For this review, take the finished solid that the model builds, in its own axes (mm). Coordinates: 2 decimals unless noted, no trailing zeros. Loops run counter-clockwise (first coordinate to the right, second up) from the corner with the lowest first, then second, coordinate; pieces in that order, holes last. Notation, with made-up numbers: (55.5, -18.5) -> (70.5, -18.5) arc R17 ccw to (70.5, -11.5) -> close; hole circle Ø5 at (-28.75, -33.75). An arc over 180 degrees is marked (long way). Answer in a Markdown table with one row per item.
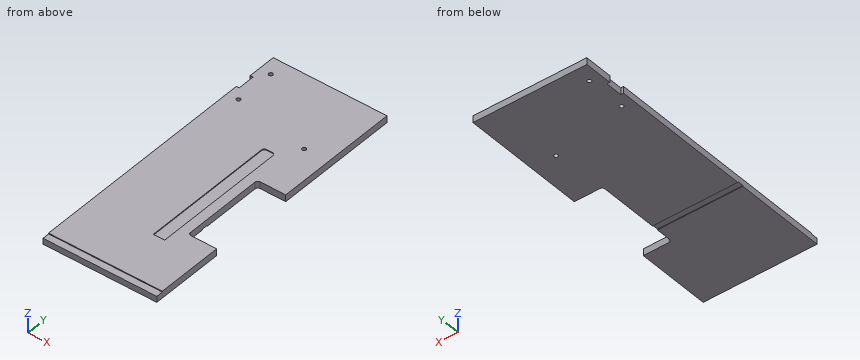
from build123d import *

# Parameters (mm, degrees)
SKETCH_1_W          = 200
SKETCH_1_H          = 500
EXTRUDE_1_DEPTH     = 6
SKETCH_2_W          = 200
SKETCH_2_H          = 11
CUT_EXTRUDE_1_DEPTH = 1.5
CUT_EXTRUDE_2_REACH = 271.526
SKETCH_3_W          = 5
SKETCH_3_H          = 30
CUT_EXTRUDE_3_REACH = 271.526
SKETCH_4_R          = 3.5
SKETCH_5_W          = 20
SKETCH_5_H          = 240
CUT_EXTRUDE_4_DEPTH = 1.5
FILLET_1_R          = 5
CUT_EXTRUDE_5_REACH = 271.526
SKETCH_6_W          = 50
SKETCH_6_H          = 150
FILLET_2_R          = 5
SKETCH_7_W          = 200
SKETCH_7_H          = 12
CUT_EXTRUDE_6_DEPTH = 1.5


with BuildPart() as part:
    # 草图1 → 凸台-拉伸1 (new, symmetric)
    with BuildSketch(Plane.XY):
        Rectangle(SKETCH_1_W, SKETCH_1_H)
    extrude(amount=EXTRUDE_1_DEPTH, both=True)

    # 草图2 → 切除-拉伸1 (cut)
    with BuildSketch(Plane.XY.offset(-6)):
        with Locations((0, -83.5)):
            Rectangle(SKETCH_2_W, SKETCH_2_H)
    extrude(amount=CUT_EXTRUDE_1_DEPTH, mode=Mode.SUBTRACT)

    # 草图3 → 切除-拉伸2 (cut, up to next)
    with BuildSketch(Plane.XY.offset(6), mode=Mode.PRIVATE) as cut_extrude_2_sk1:
        with Locations((-97.5, 185)):
            Rectangle(SKETCH_3_W, SKETCH_3_H)
    cut_extrude_2_tool1 = extrude(cut_extrude_2_sk1.sketch, amount=-CUT_EXTRUDE_2_REACH, mode=Mode.PRIVATE) & part.part
    add(cut_extrude_2_tool1.solids().sort_by_distance((-97.5, 185, 6))[0], mode=Mode.SUBTRACT)

    # 草图4 → 切除-拉伸3 (cut, up to next)
    with BuildSketch(Plane.XY.offset(6), mode=Mode.PRIVATE) as cut_extrude_3_sk1:
        with Locations((-80, 220)):
            Circle(SKETCH_4_R)
    cut_extrude_3_tool1 = extrude(cut_extrude_3_sk1.sketch, amount=-CUT_EXTRUDE_3_REACH, mode=Mode.PRIVATE) & part.part
    # 草图4 → 切除-拉伸3 (cut, up to next)
    with BuildSketch(Plane.XY.offset(6), mode=Mode.PRIVATE) as cut_extrude_3_sk2:
        with Locations((-80, 150)):
            Circle(SKETCH_4_R)
    cut_extrude_3_tool2 = extrude(cut_extrude_3_sk2.sketch, amount=-CUT_EXTRUDE_3_REACH, mode=Mode.PRIVATE) & part.part
    # 草图4 → 切除-拉伸3 (cut, up to next)
    with BuildSketch(Plane.XY.offset(6), mode=Mode.PRIVATE) as cut_extrude_3_sk3:
        with Locations((57, 123)):
            Circle(SKETCH_4_R)
    cut_extrude_3_tool3 = extrude(cut_extrude_3_sk3.sketch, amount=-CUT_EXTRUDE_3_REACH, mode=Mode.PRIVATE) & part.part
    add(cut_extrude_3_tool1.solids().sort_by_distance((-80, 220, 6))[0], mode=Mode.SUBTRACT)
    add(cut_extrude_3_tool2.solids().sort_by_distance((-80, 150, 6))[0], mode=Mode.SUBTRACT)
    add(cut_extrude_3_tool3.solids().sort_by_distance((57, 123, 6))[0], mode=Mode.SUBTRACT)

    # 草图5 → 切除-拉伸4 (cut)
    with BuildSketch(Plane(origin=(0, 0, 6), x_dir=(-1, 0, 0), z_dir=(0, 0, -1))):
        with Locations((-23, -30)):
            Rectangle(SKETCH_5_W, SKETCH_5_H)
    extrude(amount=CUT_EXTRUDE_4_DEPTH, mode=Mode.SUBTRACT)

    # 圆角1
    fillet_1_edges = [part.edges().sort_by_distance(p)[0] for p in [
        (33, 90, 5.25),
        (13, 90, 5.25),
    ]]
    fillet(fillet_1_edges, radius=FILLET_1_R)

    # 草图6 → 切除-拉伸5 (cut, up to next)
    with BuildSketch(Plane(origin=(0, 0, -6), x_dir=(-1, 0, 0), z_dir=(0, 0, -1)), mode=Mode.PRIVATE) as cut_extrude_5_sk1:
        with Locations((-75, -45)):
            Rectangle(SKETCH_6_W, SKETCH_6_H)
    cut_extrude_5_tool1 = extrude(cut_extrude_5_sk1.sketch, amount=-CUT_EXTRUDE_5_REACH, mode=Mode.PRIVATE) & part.part
    add(cut_extrude_5_tool1.solids().sort_by_distance((75, -45, -6))[0], mode=Mode.SUBTRACT)

    # 圆角2
    fillet_2_edges = [part.edges().sort_by_distance(p)[0] for p in [
        (50, 30, 0),
        (50, -120, 0),
    ]]
    fillet(fillet_2_edges, radius=FILLET_2_R)

    # 草图7 → 切除-拉伸6 (cut)
    with BuildSketch(Plane.XY.offset(6)):
        with Locations((0, -244)):
            Rectangle(SKETCH_7_W, SKETCH_7_H)
    extrude(amount=-CUT_EXTRUDE_6_DEPTH, mode=Mode.SUBTRACT)


solid = part.part
Item 1: Take a section at C-C, the plane y = -72. State the section outline as (x, z) points, and give its area (3 significant figures).
Worked answers:
| item | result |
|---|---|
| outline | (-100, -6) -> (50, -6) -> (50, 6) -> (33, 6) -> (33, 4.5) -> (13, 4.5) -> (13, 6) -> (-100, 6) -> close |
| area | 1,770 mm² |
Item 2: For L1, parallel to Y at x = -80, z = 2.5; L2, parallel to Y at x = 74.5, z = 4; L3, parallel to X at y = 220, z = -2.5, list the stretches that pass through material, from the lowest coordinate up.
Worked answers:
| item | result |
|---|---|
| L1 | -250 to 146.5, 153.5 to 216.5, 223.5 to 250 |
| L2 | -250 to -120, 30 to 250 |
| L3 | -100 to -83.5, -76.5 to 100 |
Item 3: Take a section at A-A, the plane x = 77. State the section outline as (y, z) points.
Worked answers:
| item | result |
|---|---|
| outline | (-250, -6) -> (-120, -6) -> (-120, 6) -> (-238, 6) -> (-238, 4.5) -> (-250, 4.5) -> close; (30, -6) -> (250, -6) -> (250, 6) -> (30, 6) -> close |
Item 4: Take a section at B-B, the plane z = -1.25. State the section outline as (x, y) points, and give its area (3 significant figures).
Worked answers:
| item | result |
|---|---|
| outline | (-100, -250) -> (100, -250) -> (100, -120) -> (55, -120) arc R5 cw to (50, -115) -> (50, 25) arc R5 cw to (55, 30) -> (100, 30) -> (100, 250) -> (-100, 250) -> (-100, 200) -> (-95, 200) -> (-95, 170) -> (-100, 170) -> close; hole circle Ø7 at (-80, 150); hole circle Ø7 at (-80, 220); hole circle Ø7 at (57, 123) |
| area | 92,200 mm² |
Item 5: Take a section at D-D, the plane y = 187. State the section outline as (x, z) points.
Worked answers:
| item | result |
|---|---|
| outline | (-95, -6) -> (100, -6) -> (100, 6) -> (-95, 6) -> close |
Item 6: Insertion check: pin 1 (3.5 mm diameter, centred on y = 191.5, z = 0, fed in from -X); pin 2 (1.2 mm diameter, centred on y = -25.5, z = 5, fed in from +X). Each pin has a flat end and moves straight along its axis. Give the tip position at first contact, or say it passes through.
Worked answers:
| item | result |
|---|---|
| pin 1 | x = -95 |
| pin 2 | x = 50 |
